Could you check a few things on this model? Use its own coordinates, in mm. A direction names the side the tool comes from. Give positions to 0.01 mm unless a question says otherwise; leave off trailing zeros. Order: outer loops, then holes, each group sorted by start corner. A loop starts at its lowest first (then second) coordinate and runs counter-clockwise, first axis right, second up. Notation, with made-up numbers: (55.25, 57) - (88.25, 57) arc R21 cw to (88.25, 88) - close; hole circle Ø11 at (-26, -30). An arc over 180 degrees is marked (long way). Put each result on its own line as item: value.
from build123d import *

# Parameters (mm, degrees)
SKETCH_1_W             = 75
SKETCH_1_H             = 120
EXTRUDE_1_DEPTH        = 5
SKETCH_2_W             = 55
SKETCH_2_H             = 100
CUT_EXTRUDE_1_DEPTH    = 10
FILLET_1_R             = 15
FILLET_2_R             = 10
HOLE_WIZARD_M4_1_D     = 3.3
HOLE_WIZARD_M4_1_DEPTH = 10.1
HOLE_WIZARD_M4_1_TIP   = 0.991420021
HOLE_WIZARD_M4_2_D     = 3.3
HOLE_WIZARD_M4_2_DEPTH = 10.1
HOLE_WIZARD_M4_2_TIP   = 0.991420021


with BuildPart() as part:
    # 草图1 → 凸台-拉伸1 (new, symmetric)
    with BuildSketch(Plane(origin=(0, 0, 0), x_dir=(1, 0, 0), z_dir=(0, 1, 0))):
        Rectangle(SKETCH_1_W, SKETCH_1_H)
    extrude(amount=EXTRUDE_1_DEPTH, both=True)

    # 草图2 → 切除-拉伸1 (cut)
    with BuildSketch(Plane(origin=(0, 5, 0), x_dir=(1, 0, 0), z_dir=(0, 1, 0))):
        with Locations((-10, 10)):
            Rectangle(SKETCH_2_W, SKETCH_2_H)
    extrude(amount=-CUT_EXTRUDE_1_DEPTH, mode=Mode.SUBTRACT)

    # 圆角1
    fillet_1_edges = [part.edges().sort_by_distance(p)[0] for p in [
        (17.5, 0, 40),
    ]]
    fillet(fillet_1_edges, radius=FILLET_1_R)

    # 圆角2
    fillet_2_edges = [part.edges().sort_by_distance(p)[0] for p in [
        (17.5, 0, -60),
        (-37.5, 0, 40),
    ]]
    fillet(fillet_2_edges, radius=FILLET_2_R)

    # M4 螺纹孔1
    with Locations(Plane.XY.offset(60)):
        with Locations((-30, 0), (20, 0)):
            Hole(HOLE_WIZARD_M4_1_D / 2, depth=HOLE_WIZARD_M4_1_DEPTH)
            with Locations((0, 0, -(HOLE_WIZARD_M4_1_DEPTH + HOLE_WIZARD_M4_1_TIP / 2))):  # 118° drill point
                Cone(0, HOLE_WIZARD_M4_1_D / 2, HOLE_WIZARD_M4_1_TIP, mode=Mode.SUBTRACT)

    # M4 螺纹孔2
    with Locations(Plane(origin=(37.5, 0, 0), x_dir=(0, 0, -1), z_dir=(1, 0, 0))):
        with Locations((-27.5, 0), (52.5, 0)):
            Hole(HOLE_WIZARD_M4_2_D / 2, depth=HOLE_WIZARD_M4_2_DEPTH)
            with Locations((0, 0, -(HOLE_WIZARD_M4_2_DEPTH + HOLE_WIZARD_M4_2_TIP / 2))):  # 118° drill point
                Cone(0, HOLE_WIZARD_M4_2_D / 2, HOLE_WIZARD_M4_2_TIP, mode=Mode.SUBTRACT)


solid = part.part
1) We'd pull the mould along X, two halves only. Please class faces 5 (the cylindrical face through (32.38, 0.07, -54.15)), 6 (the cylindrical face through (12.99, -0.07, 35.72)), 7 (the conical face through (20.3, -0.1, 49.1)): pulls with the +X half, pulls with the -X half, needs draft (parallel to the pull), parting line crosses it, or undercut.
Filled in:
face 5: needs draft
face 6: pulls with the -X half
face 7: undercut
2) I'm going to push flat-ended pins straight in: pin 1 (3 mm diameter, centred on x = -19.5, y = -0.5, fed in from -Z); pin 2 (4 mm diameter, centred on x = 5.5, y = 2, fed in from -Z); pin 3 (3 mm diameter, centred on y = 2.5, z = -11, fed in from -X); pin 4 (4.5 mm diameter, centred on x = 20, y = 0, fed in from +Z). Where does each tip first touch, or does it pass through?
Filled in:
pin 1: stops at z = 40
pin 2: stops at z = 39.14
pin 3: stops at x = 17.5
pin 4: stops at z = 60
3) If I drill on line 1 (X direction, y = 0, z = 53.5); line 2 (Z direction, x = 32, y = 0); line 3 (Y direction, x = 20, z = 58), over which ranges is the centre line in solid material (lowest first)? Write a range as [from, to].
Filled in:
line 1: x = [-37.5, -31.65], [-28.35, 18.35], [21.65, 37.5]
line 2: z = [-60, -54.15], [-50.85, 25.85], [29.15, 60]
line 3: y = [-5, -1.65], [1.65, 5]
4) Suppose I cut it at C-C, the plane x = -20. List the corners of the cut face in (y, z) for me, and give its area (3 significant figures).
Filled in:
outline: (-5, 40) - (5, 40) - (5, 60) - (-5, 60) - close
area: 200 mm^2
5) Suppose I cut it at A-A, the plane y = -3.5. List the corners of the cut face in (x, z) for me, and give its area (3 significant figures).
Filled in:
outline: (-37.5, 50) arc R10 ccw to (-27.5, 40) - (2.5, 40) arc R15 cw to (17.5, 25) - (17.5, -50) arc R10 ccw to (27.5, -60) - (37.5, -60) - (37.5, 60) - (-37.5, 60) - close
area: 3,510 mm^2
6) Which directions (+Z, -Z, +X, -X, +Y, -Y) give clear straight access to the entire face, cutting with the end or side of a thin tool? Please do faces 1 (the cylindrical face through (32.38, 0.07, 25.85)), 2 (the flat face through (17.5, 0, -12)), 3 (the cylindrical face through (-28.35, 0.07, 54.88)), 4 (the flat face through (-1, 0, 60)).
Filled in:
face 1: +X
face 2: -Z, -X, +Y, -Y
face 3: +Z
face 4: +Z, +X, -X, +Y, -Y
7) Suppose I cut it at B-B, the plane z = 11.5. List the corners of the cut face in (x, y) for me, and give its area (3 significant figures).
Filled in:
outline: (17.5, -5) - (37.5, -5) - (37.5, 5) - (17.5, 5) - close
area: 200 mm^2
